The listing builds one solid part. Answer for the finished solid, in the listing's coordinates (mm). Face numbers are marked on the shaded views. Coordinates: 2 decimals unless noted, no trailing zeros. Loops run counter-clockwise (first coordinate to the right, second up) from the corner with the lowest first, then second, coordinate; pieces in that order, holes last. Notation, with made-up numbers: (42.5, 12) -> (82.5, 12) arc R18 cw to (82.5, 34) -> close; hole circle Ø6 at (56.25, -21.75). An arc over 180 degrees is marked (long way). Answer in a Markdown table with one row per item.
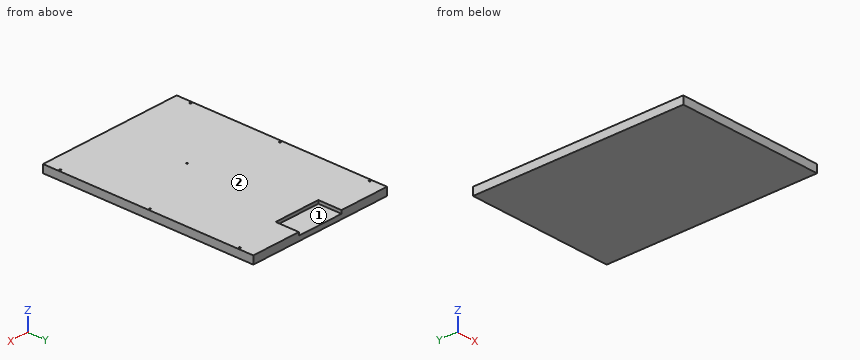
```python
from build123d import *

# Parameters (mm, degrees)
SKETCH_1_W            = 940
SKETCH_1_H            = 1360
EXTRUDE_1_DEPTH       = 50
SKETCH_2_R            = 5
SKETCH_2_R_2          = 5.5
SKETCH_2_W            = 300
SKETCH_2_H            = 300
CUT_EXTRUDE_986_DEPTH = 20


with BuildPart() as part:
    # 草图1 → 凸台-拉伸1 (new body)
    with BuildSketch(Plane.XY):
        Rectangle(SKETCH_1_W, SKETCH_1_H)
    extrude(amount=EXTRUDE_1_DEPTH)

    # 草图2 → Cut-Extrude 986 (cut)
    with BuildSketch(Plane.XY.offset(50)):
        with Locations((0, -180)):
            Circle(SKETCH_2_R)
        with Locations((457.5, -580)):
            Circle(SKETCH_2_R_2)
        with Locations((457.5, 0)):
            Circle(SKETCH_2_R_2)
        with Locations((457.5, 580)):
            Circle(SKETCH_2_R_2)
        with Locations(Location((-457.5, 580, 0), (0, 0, 180))):
            Circle(SKETCH_2_R_2)
        with Locations(Location((-457.5, 0, 0), (0, 0, 180))):
            Circle(SKETCH_2_R_2)
        with Locations(Location((-457.5, -580, 0), (0, 0, 180))):
            Circle(SKETCH_2_R_2)
        with Locations((0, 680)):
            Rectangle(SKETCH_2_W, SKETCH_2_H)
    extrude(amount=-CUT_EXTRUDE_986_DEPTH, mode=Mode.SUBTRACT)


solid = part.part
```
Item 1: Flat-ended cylindrical pins translate along their axes: pin 1 Ø16 at (x, z) = (34, 41.5) entering from +Y; pin 2 Ø9 at (x, y) = (457.5, 580) entering from +Z. Find the tip coordinate at first contact, or state that the pin passes through.
Findings below:
| item | result |
|---|---|
| pin 1 | stops at y = 530 |
| pin 2 | stops at z = 30 |
Item 2: A cutting plane is placed at A-A, the plane x = -134.5. Determine the outline of the cut face in (y, z).
Findings below:
| item | result |
|---|---|
| outline | (-680, 0) -> (680, 0) -> (680, 30) -> (530, 30) -> (530, 50) -> (-680, 50) -> close |
Item 3: Find the intervals of material crossed by probe 1 along X at (y, z) = (580, 43); probe 2 along Y at (x, z) = (-457.5, 37); probe 3 along X at (y, z) = (-580, 36.5), in increasing order.
Findings below:
| item | result |
|---|---|
| probe 1 | x = -470 to -463, -452 to -150, 150 to 452, 463 to 470 |
| probe 2 | y = -680 to -585.5, -574.5 to -5.5, 5.5 to 574.5, 585.5 to 680 |
| probe 3 | x = -470 to -463, -452 to 452, 463 to 470 |
Item 4: Determine the mould class of the marked faces 1 and 2 for opening direction X: +X half, -X half, draft (parallel to the pull), parting line (faces both ways), or undercut.
Findings below:
| item | result |
|---|---|
| face 1 | undercut |
| face 2 | draft |
